Input: part model. Units: mm. Frame: model coordinates. Face numbers are marked on the shaded views. A direction names the side the tool comes from. Give positions to 0.01 mm unless a question says otherwise; leave off trailing zeros. Loops run counter-clockwise (first coordinate to the right, second up) from the corner with the lowest first, then second, coordinate; pieces in that order, holes last. Notation, with made-up numbers: (57, 1) - (83, 1) arc R24 ccw to (83, 34) - close; hole circle Ø2 at (72.25, -4.75). An arc over 180 degrees is marked (long way). Answer as a JSON object with one key per item and string values. Group by question number.
(1) Pin query (flat end, axial travel): P1, Ø5, axis at x = 34, z = 82.5, coming from the -Y side. Return the tip coordinate at first contact, or that it passes through.
(2) Section query A-A (y = 34). Return loops of the section in (x, z), plus the area to 3 significant figures.
(3) Access query for the marked faces 5 and 6. Directions: +Z, -Z, +X, -X, +Y, -Y. A direction counts if a zero-diameter tool reaches every point of the face in a straight line with its end or side. Return the directions, or none.
(4) Mould query, pull axis Z, two halves, no side actions, for the marked faces 1, 2, 3 and 4. Classes: +Z half, -Z half, draft (parallel to the pull), parting line (faces both ways), or undercut.
(5) Material intervals for L1, parallel to Z at x = 64.5, y = 36.5; L2, parallel to Y at x = 85.5, z = 38; L3, parallel to Y at x = 34, z = 94, sorted ascending.
(6) Section query D-D (z = 39). Return loops of the section in (x, y), plus the area to 3 significant figures.
(7) Section query C-C (y = 26.5). Return loops of the section in (x, z).
(8) Section query B-B (x = 89.5). Return loops of the section in (y, z).
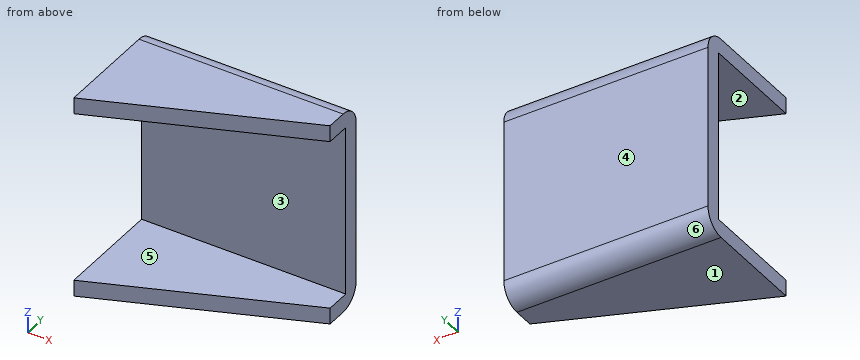
```python
from build123d import *

# Parameters (mm, degrees)
EXTRUDE_1_DEPTH = 100
SHELL_1_T       = -8
FILLET_1_R      = 10
FILLET_2_R      = 10


with BuildPart() as part:
    # 草图1 → 凸台-拉伸1 (new body)
    with BuildSketch(Plane.XY):
        Polygon((0, 0), (0, 60), (100, 60), (100, 40), align=None)
    extrude(amount=EXTRUDE_1_DEPTH)

    # 抽壳1
    shell_1_openings = [part.faces().sort_by_distance(p)[0] for p in [
        (0, 30, 50),
        (100, 50, 50),
        (50, 20, 50),
    ]]
    offset(amount=SHELL_1_T, openings=shell_1_openings, kind=Kind.INTERSECTION)

    # 圆角1
    fillet_1_edges = [part.edges().sort_by_distance(p)[0] for p in [
        (50, 60, 100),
    ]]
    fillet(fillet_1_edges, radius=FILLET_1_R)

    # 圆角2
    fillet_2_edges = [part.edges().sort_by_distance(p)[0] for p in [
        (50, 60, 0),
    ]]
    fillet(fillet_2_edges, radius=FILLET_2_R)


solid = part.part
```
Recorded:
{
 "1": {"P1": "stops at y = 52"},
 "2": {"outline": "(0, 0) - (85, 0) - (85, 8) - (0, 8) - close; (0, 92) - (85, 92) - (85, 100) - (0, 100) - close", "area": "1,360 mm^2"},
 "3": {"face 5": "+X, -X, -Y", "face 6": "-Z, +X, -X, +Y"},
 "4": {"face 1": "-Z half", "face 2": "undercut", "face 3": "undercut", "face 4": "draft"},
 "5": {"L1": "z = 0 to 8, 92 to 100", "L2": "y = 52 to 60", "L3": "y = 13.6 to 59.17"},
 "6": {"outline": "(0, 52) - (100, 52) - (100, 60) - (0, 60) - close", "area": "800 mm^2"},
 "7": {"outline": "(0, 0) - (66.25, 0) - (66.25, 8) - (0, 8) - close; (0, 92) - (66.25, 92) - (66.25, 100) - (0, 100) - close"},
 "8": {"outline": "(35.8, 0) - (50, 0) arc R10 ccw to (60, 10) - (60, 90) arc R10 ccw to (50, 100) - (35.8, 100) - (35.8, 92) - (52, 92) - (52, 8) - (35.8, 8) - close"}
}
